```python
from build123d import *

# Parameters (mm, degrees)
SKETCH1_W           = 50
SKETCH1_H           = 40
BOSS_EXTRUDE1_DEPTH = 8
SKETCH3_W           = 20
SKETCH3_H           = 52
BOSS_EXTRUDE2_DEPTH = 8
SKETCH2_R           = 5
CUT_EXTRUDE1_DEPTH  = 69.410525506
CHAMFER2_SIZE       = 1
SKETCH4_W           = 20
SKETCH4_H           = 8
BOSS_EXTRUDE3_DEPTH = 12
CHAMFER4_SIZE       = 1
FILLET1_R           = 2
SKETCH5_W           = 8
SKETCH5_H           = 40
BOSS_EXTRUDE4_DEPTH = 20
CHAMFER5_SIZE       = 1
SKETCH6_R           = 2.5
CUT_EXTRUDE2_DEPTH  = 1
CUT_EXTRUDE3_START  = -1
SKETCH7_R           = 2.5
CUT_EXTRUDE3_DEPTH  = 1


with BuildPart() as part:
    # Sketch1 → Boss-Extrude1 (new body)
    with BuildSketch(Plane(origin=(0, 0, 0), x_dir=(1, 0, 0), z_dir=(0, 1, 0))):
        with Locations((25, -20)):
            Rectangle(SKETCH1_W, SKETCH1_H)
    extrude(amount=BOSS_EXTRUDE1_DEPTH)

    # Sketch3 → Boss-Extrude2 (add)
    with BuildSketch(Plane(origin=(0, 8, 0), x_dir=(1, 0, 0), z_dir=(0, 1, 0))):
        with Locations((40, -20)):
            Rectangle(SKETCH3_W, SKETCH3_H)
    extrude(amount=-BOSS_EXTRUDE2_DEPTH)

    # Sketch2 → Cut-Extrude1 (cut, through all)
    with BuildSketch(Plane.XZ):
        with Locations(Location((40, 20, 0), (0, 0, 270))):
            Circle(SKETCH2_R)
    extrude(amount=-CUT_EXTRUDE1_DEPTH, mode=Mode.SUBTRACT)

    # Chamfer2
    chamfer2_edges = [part.edges().sort_by_distance(p)[0] for p in [
        (40, 8, 25),
        (40, 0, 25),
    ]]
    chamfer(chamfer2_edges, length=CHAMFER2_SIZE)

    # Sketch4 → Boss-Extrude3 (add)
    with BuildSketch(Plane(origin=(0, 0, 0), x_dir=(1, 0, 0), z_dir=(0, 1, 0))):
        with Locations((40, -42)):
            Rectangle(SKETCH4_W, SKETCH4_H)
        with Locations((40, 2)):
            Rectangle(SKETCH4_W, SKETCH4_H)
    extrude(amount=-BOSS_EXTRUDE3_DEPTH)

    # Chamfer4
    chamfer4_edges = [part.edges().sort_by_distance(p)[0] for p in [
        (30, -12, 42),
        (50, -12, 42),
        (30, -12, -2),
        (50, -12, -2),
    ]]
    chamfer(chamfer4_edges, length=CHAMFER4_SIZE)

    # Fillet1
    fillet1_edges = [part.edges().sort_by_distance(p)[0] for p in [
        (30, 4, 40),
        (30, 4, 0),
    ]]
    fillet(fillet1_edges, radius=FILLET1_R)

    # Sketch5 → Boss-Extrude4 (add)
    with BuildSketch(Plane(origin=(0, 8, 0), x_dir=(1, 0, 0), z_dir=(0, 1, 0))):
        with Locations((4, -20)):
            Rectangle(SKETCH5_W, SKETCH5_H)
    extrude(amount=BOSS_EXTRUDE4_DEPTH)

    # Chamfer5
    chamfer5_edges = [part.edges().sort_by_distance(p)[0] for p in [
        (4, 28, 40),
        (4, 28, 0),
    ]]
    chamfer(chamfer5_edges, length=CHAMFER5_SIZE)

    # Sketch6 → Cut-Extrude2 (cut)
    with BuildSketch(Plane.XY.offset(2)):
        with Locations((44, -7)):
            Circle(SKETCH6_R)
        with Locations((36, -7)):
            Circle(SKETCH6_R)
    extrude(amount=-CUT_EXTRUDE2_DEPTH, mode=Mode.SUBTRACT)

    # Sketch7 → Cut-Extrude3 (cut)
    with BuildSketch(Plane(origin=(0, 0, 38), x_dir=(-1, 0, 0), z_dir=(0, 0, -1)).offset(CUT_EXTRUDE3_START)):
        with Locations(Location((-36, -7, 0), (0, 0, 180))):
            Circle(SKETCH7_R)
        with Locations(Location((-44, -7, 0), (0, 0, 180))):
            Circle(SKETCH7_R)
    extrude(amount=CUT_EXTRUDE3_DEPTH, mode=Mode.SUBTRACT)


solid = part.part
```
Can you work these out from the model? Positions are in its coordinate system, mm. A direction names the side the tool comes from. Round coordinates to 2 decimals unless told otherwise and drop trailing zeros. Loops run counter-clockwise (first coordinate to the right, second up) from the corner with the lowest first, then second, coordinate; pieces in that order, holes last. Notation, with made-up numbers: (-1.75, 66.25) -> (36.25, 66.25) arc R26 cw to (36.25, 102.25) -> close; hole circle Ø1 at (76, -37.5). An arc over 180 degrees is marked (long way). One line per item, written item: value. Start each with the question number.
1. If we section it at C-C, the plane x = 40: Write out the boundary of the cut face in (y, z).
2. For pin 1 (1 mm diameter, centred on x = 6.5, z = 21, fed in from -Y); pin 2 (2.5 mm diameter, centred on y = 3, z = 44, fed in from -X); pin 3 (8 mm diameter, centred on x = 18.5, y = 7.5, fed in from +Z), each with a flat end and sliding along its axis, tell me the tip position at first contact or that it passes through.
3. If I drill on probe 1 along X at (y, z) = (-7, 38.55); probe 2 along Y at (x, z) = (13.5, 8), over which ranges is the centre line in solid material (lowest first)?
4. For faces 4 (the flat face through (40, -6, 2)), 5 (the flat face through (44, -7, 39)), 6 (the flat face through (30, -3, -3)), 7 (the flat face through (11, 7, 0)), which set-ups out of +Z, -Z, +X, -X, +Y, -Y let a thin tool reach every point of the face, with its end or its side?
5. If we mould it in two halves opening along X, with no side actions, what happens to faces 1 (the flat face through (29, 8, 20)), 2 (the cylindrical face through (29.43, 3.94, 40.6)), 3 (the flat face through (44, -7, 1))? For each: pulls with the +X half, pulls with the -X half, needs draft (parallel to the pull), parting line crosses it, or undercut.
6. If we section it at B-B, the plane y = -7: Write out the boundary of the cut face in (x, z).
7. If we section it at A-A, the plane z = 20: Write out the boundary of the cut face in (x, y), then the cut area to 3 significant figures.
8. If we section it at D-D, the plane y = 3: Write out the boundary of the cut face in (x, z), then the cut area to 3 significant figures.
Calculated:
1. outline: (-12, -6) -> (8, -6) -> (8, 14) -> (7, 15) -> (1, 15) -> (0, 14) -> (0, 2) -> (-12, 2) -> close; (-12, 38) -> (0, 38) -> (0, 26) -> (1, 25) -> (7, 25) -> (8, 26) -> (8, 46) -> (-12, 46) -> close
2. pin 1: stops at y = 0
2. pin 2: stops at x = 30
2. pin 3: stops at z = 40
3. probe 1: x = 30 to 33.5, 38.5 to 41.5, 46.5 to 50
3. probe 2: y = 0 to 8
4. face 4: +X, -X, -Y
4. face 5: none
4. face 6: -Z, -X, -Y
4. face 7: -Z, -X, +Y, -Y
5. face 1: needs draft
5. face 2: pulls with the -X half
5. face 3: undercut
6. outline: (30, -6) -> (50, -6) -> (50, 2) -> (46.5, 2) -> (46.5, 1) -> (41.5, 1) -> (41.5, 2) -> (38.5, 2) -> (38.5, 1) -> (33.5, 1) -> (33.5, 2) -> (30, 2) -> close; (30, 38) -> (33.5, 38) -> (33.5, 39) -> (38.5, 39) -> (38.5, 38) -> (41.5, 38) -> (41.5, 39) -> (46.5, 39) -> (46.5, 38) -> (50, 38) -> (50, 46) -> (30, 46) -> close
7. outline: (0, 0) -> (34, 0) -> (35, 1) -> (35, 7) -> (34, 8) -> (8, 8) -> (8, 28) -> (0, 28) -> close; (45, 1) -> (46, 0) -> (50, 0) -> (50, 8) -> (46, 8) -> (45, 7) -> close
7. area: 478 mm²
8. outline: (0, 0) -> (28, 0) arc R2 cw to (30, -2) -> (30, -6) -> (50, -6) -> (50, 46) -> (30, 46) -> (30, 42) arc R2 cw to (28, 40) -> (0, 40) -> close; hole circle Ø10 at (40, 20)
8. area: 2,160 mm²
